Work out the finished part from the listing and answer in its coordinate system (mm). A direction names the side the tool comes from. Coordinates: 2 decimals unless noted, no trailing zeros. Write each loop counter-clockwise with the first axis right and the second up, starting at its lowest first coordinate (ties: lowest second). Pieces come first, ordered by that corner, then holes. Notation, with made-up numbers: (37, 36.25) - (80, 36.25) arc R21 cw to (80, 75.25) - close; hole circle Ø2 at (8.5, 49.5). An arc over 180 degrees is marked (long way). Use one line per item in the form item = value. Start each with the question number.
Item 1: A cutting plane is placed at B-B (x = 0). Write down the section's boundary in (y, z), then the cut area to 3 significant figures.
Item 2: A cutting plane is placed at D-D (y = 4.25). Write down the section's boundary in (x, z), then the cut area to 3 significant figures.
Item 3: Consider probe 1 along Y at (x, z) = (-3.25, 0.75); probe 2 along Y at (x, z) = (2.25, 0.5); probe 3 along X at (y, z) = (11.5, 0). Determine where each line is inside the solid, lowest interval first.
Item 4: For faces 1 (the cylindrical face through (-0.05, 18.83, 1.25)), 2 (the flat face through (0, 24, 0)), determine the directions among +Z, -Z, +X, -X, +Y, -Y from which every point of the face is accessible in a straight line to the end or side of a thin tool.
Item 5: Given pin 1 (3 mm diameter, centred on y = 21, z = 0.5, fed in from +X), flat-ended and moving along its own axis, determine where the tip first touches the part or whether it passes through.
Item 6: A cutting plane is placed at C-C (y = 11). Write down the section's boundary in (x, z).
Item 7: A cutting plane is placed at A-A (z = 0). Write down the section's boundary in (x, y), then the cut area to 3 significant figures.
from build123d import *

# Parameters (mm, degrees)
CHAMFER_1_SIZE = 0.5
FILLET_1_R     = 1
CHAMFER_2_SIZE = 0.2


with BuildPart() as part:
    # 草图1 → 旋转1 (revolve)
    with BuildSketch(Plane.XY, mode=Mode.PRIVATE) as revolve_1_sk:
        Polygon((1.25, 24), (1.25, 13), (3, 13), (3, 4.5), (4, 4.5), (4, 0), (0, 0), (0, 24), align=None)
    revolve(revolve_1_sk.sketch.rotate(Axis((0, -0.524377328, 0), (0, 1, 0)), 90), axis=Axis((0, -0.524377328, 0), (0, 1, 0)))

    # 倒角1
    chamfer_1_edges = [part.edges().sort_by_distance(p)[0] for p in [
        (0, 0, 4),
        (0, 4.5, 4),
    ]]
    chamfer(chamfer_1_edges, length=CHAMFER_1_SIZE)

    # 圆角1
    fillet_1_edges = [part.edges().sort_by_distance(p)[0] for p in [
        (0, 13, 1.25),
    ]]
    fillet(fillet_1_edges, radius=FILLET_1_R)

    # 倒角2
    chamfer_2_edges = [part.edges().sort_by_distance(p)[0] for p in [
        (0, 24, 1.25),
    ]]
    chamfer(chamfer_2_edges, length=CHAMFER_2_SIZE)


solid = part.part
Answer:
q1.outline = (0, -3.5) - (0.5, -4) - (4, -4) - (4.5, -3.5) - (4.5, -3) - (13, -3) - (13, -2.25) arc R1 cw to (14, -1.25) - (23.8, -1.25) - (24, -1.05) - (24, 1.05) - (23.8, 1.25) - (14, 1.25) arc R1 cw to (13, 2.25) - (13, 3) - (4.5, 3) - (4.5, 3.5) - (4, 4) - (0.5, 4) - (0, 3.5) - close
q1.area = 114 mm²
q2.outline = circle Ø7.5 at (0, 0)
q2.area = 44.2 mm²
q3.probe_1 = 0 to 4.5
q3.probe_2 = 0 to 13
q3.probe_3 = -3 to 3
q4.face_1 = +Y
q4.face_2 = +Z, -Z, +X, -X, +Y
q5.pin_1 = 1.25
q6.outline = circle Ø6 at (0, 0)
q7.outline = (-4, 0.5) - (-3.5, 0) - (3.5, 0) - (4, 0.5) - (4, 4) - (3.5, 4.5) - (3, 4.5) - (3, 13) - (2.25, 13) arc R1 cw to (1.25, 14) - (1.25, 23.8) - (1.05, 24) - (-1.05, 24) - (-1.25, 23.8) - (-1.25, 14) arc R1 cw to (-2.25, 13) - (-3, 13) - (-3, 4.5) - (-3.5, 4.5) - (-4, 4) - close
q7.area = 114 mm²
